from build123d import *

# Parameters (mm, degrees)
SKETCH1_R               = 60
SKETCH1_R_2             = 30
BOSS_EXTRUDE1_DEPTH     = 14
CUT_EXTRUDE1_DEPTH      = 87
CUT_EXTRUDE1_DEPTH_BACK = 87
SKETCH2_OUTSIDE_W       = 156.4
SKETCH2_OUTSIDE_H       = 156.4
SKETCH2_OUTSIDE_W_2     = 160
SKETCH2_OUTSIDE_H_2     = 115
SKETCH3_R               = 6.5
CUT_EXTRUDE2_DEPTH      = 131.464554573


with BuildPart() as part:
    # Sketch1 → Boss-Extrude1 (new, symmetric)
    with BuildSketch(Plane(origin=(0, 0, 0), x_dir=(1, 0, 0), z_dir=(0, 1, 0))):
        with Locations(Location((0, 0, 0), (0, 0, 270))):
            Circle(SKETCH1_R)
        with Locations(Location((0, 0, 0), (0, 0, 270))):
            Circle(SKETCH1_R_2, mode=Mode.SUBTRACT)
    extrude(amount=BOSS_EXTRUDE1_DEPTH, both=True)

    # Sketch2 outside → Cut-Extrude1 (cut, two sides: drawn at the far end of the back side and taken through both)
    with BuildSketch(Plane(origin=(0, 0, 0), x_dir=(1, 0, 0), z_dir=(0, 1, 0)).offset(-CUT_EXTRUDE1_DEPTH_BACK)):
        Rectangle(SKETCH2_OUTSIDE_W, SKETCH2_OUTSIDE_H)
        Rectangle(SKETCH2_OUTSIDE_W_2, SKETCH2_OUTSIDE_H_2, mode=Mode.SUBTRACT)
    extrude(amount=CUT_EXTRUDE1_DEPTH + CUT_EXTRUDE1_DEPTH_BACK, mode=Mode.SUBTRACT)

    # Sketch3 → Cut-Extrude2 (cut, through all)
    with BuildSketch(Plane.XY.offset(57.5)):
        with Locations((0, 1)):
            Circle(SKETCH3_R)
    extrude(amount=-CUT_EXTRUDE2_DEPTH, mode=Mode.SUBTRACT)


solid = part.part
Can you work these out from the model? Positions are in its coordinate system, mm. Round coordinates to 2 decimals unless told otherwise and drop trailing zeros. Write each loop counter-clockwise with the first axis right and the second up, starting at its lowest first coordinate (ties: lowest second). Pieces come first, ordered by that corner, then holes. Notation, with made-up numbers: (6, 1.25) -> (28, 1.25) arc R22 cw to (28, 10.25) -> close; hole circle Ø1 at (64.25, 48). An arc over 180 degrees is marked (long way). One line per question, with ' | ' between items. Start each with the question number.
1) If we mould it in two halves opening along Y, with no side actions, what happens to faces 1 (the cylindrical face through (59.99, 0.2, 1.08)), 2 (the cylindrical face through (-5.158, -2.955, -43.196)), 3 (the flat face through (28, 14, -14))? For each: released by +Y, released by -Y, zero draft, split by the parting line, or undercut.
2) Suppose I cut it at A-A on z = 0. Write out the boundary of the cut face in (x, y).
3) Suppose I cut it at C-C on y = 1. Write out the boundary of the cut face in (x, z), then the cut area to 3 significant figures.
4) I'm going to push flat-ended pins straight in: P1, Ø1.5, axis at y = -1, z = 14.5, coming from the -X side; P2, Ø2, axis at x = 25, y = -2.5, coming from the -Z side; P3, Ø8, axis at y = -4.5, z = -13.5, coming from the -X side. Where does each tip first touch, or does it pass through?
5) Suppose I cut it at B-B on x = 0. Write out the boundary of the cut face in (y, z).
6) I need wall thicknesses on line 1 (Y direction, x = 0, z = -40); line 2 (Z direction, x = 24, y = -1.5); line 3 (Z direction, x = 25, y = 0.75). Which ranges of each line are inside material? Lowest first, please. Write a range as [from, to].
7) Suppose I cut it at D-D on x = -22.5. Write out the boundary of the cut face in (y, z), then the cut area to 3 significant figures.
Return value:
1) face 1: zero draft | face 2: undercut | face 3: released by +Y
2) outline: (-60, -14) -> (-30, -14) -> (-30, 14) -> (-60, 14) -> close; (30, -14) -> (60, -14) -> (60, 14) -> (30, 14) -> close
3) outline: (-17.14, -57.5) -> (-6.5, -57.5) -> (-6.5, -29.29) arc R30 cw to (-6.5, 29.29) -> (-6.5, 57.5) -> (-17.14, 57.5) arc R60 ccw to start; (6.5, -57.5) -> (17.14, -57.5) arc R60 ccw to (17.14, 57.5) -> (6.5, 57.5) -> (6.5, 29.29) arc R30 cw to (6.5, -29.29) -> close | area: 7,650 mm2
4) P1: stops at x = -58.4 | P2: stops at z = -54.99 | P3: stops at x = -59.24
5) outline: (-14, -57.5) -> (-5.5, -57.5) -> (-5.5, -30) -> (-14, -30) -> close; (-14, 30) -> (-5.5, 30) -> (-5.5, 57.5) -> (-14, 57.5) -> close; (7.5, -57.5) -> (14, -57.5) -> (14, -30) -> (7.5, -30) -> close; (7.5, 30) -> (14, 30) -> (14, 57.5) -> (7.5, 57.5) -> close
6) line 1: y = [-14, -5.5], [7.5, 14] | line 2: z = [-54.99, -18], [18, 54.99] | line 3: z = [-54.54, -16.58], [16.58, 54.54]
7) outline: (-14, -55.62) -> (14, -55.62) -> (14, -19.84) -> (-14, -19.84) -> close; (-14, 19.84) -> (14, 19.84) -> (14, 55.62) -> (-14, 55.62) -> close | area: 2,000 mm2
